The listing builds one solid part. Answer for the finished solid, in the listing's coordinates (mm). A direction names the side the tool comes from. Give positions to 0.01 mm unless a question says otherwise; leave off trailing zeros. Order: outer loops, then holes, each group sorted by start corner. A loop starts at its lowest first (then second) coordinate and runs counter-clockwise, first axis right, second up. Notation, with made-up numbers: (52, 15) - (72, 15) arc R24 ccw to (72, 26) - close; hole circle Ø6 at (21.5, -25.5). An arc over 180 degrees is marked (long way). Answer as a JSON object with one key per item and string values. Group by question number.
Q1. Consider line 1 (Z direction, x = -48, y = 83.75); line 2 (X direction, y = 33, z = 15); line 3 (X direction, y = 79, z = 77). Determine where each line is inside the solid, lowest interval first.
Q2. For faces 4 (the face through (-19, 89, 87)), 5 (the face through (33.289, 86.084, 20.804)), 6 (the face through (-72, 10, 78)), 7 (the face through (-80, 53, 47)), 8 (the face through (-64, 51, 47)), determine the directions among +Z, -Z, +X, -X, +Y, -Y from which every point of the face is accessible in a straight line to the end or side of a thin tool.
Q3. A cutting plane is placed at C-C, the plane y = 11.5. Give the vertices of the cut face in (x, z), and give its area (3 significant figures).
Q4. A cutting plane is placed at B-B, the plane x = 0. Give the vertices of the cut face in (y, z), and give its area (3 significant figures).
Q5. A cutting plane is placed at D-D, the plane x = 48. Give the vertices of the cut face in (y, z), and give its area (3 significant figures).
Q6. A cutting plane is placed at A-A, the plane z = 48. Give the vertices of the cut face in (x, y), and give its area (3 significant figures).
Q7. Given pin 1 (15 mm diameter, centred on x = -1.5, z = 91, fed in from +Y); pin 2 (9.5 mm diameter, centred on y = 86.5, z = 43.5, fed in from +X); pin 3 (16 mm diameter, centred on y = 26.5, z = 65.5, fed in from +X); pin 4 (6 mm diameter, centred on y = 89, z = 56.5, fed in from -X), each flat-ended and moving along its own axis, determine where each tip first touches the part or whether it passes through.
Q8. The mould has two halves that part along X. Classify faces 1 (the face through (-12, 77, 96)), 2 (the face through (-65.703, 78.014, 47.328)), 3 (the face through (-19, 89, 10)): released by +X, released by -X, zero draft, split by the parting line, or undercut.
from build123d import *

# Parameters (mm, degrees)
BRIDGE_BODY_DEPTH          = 96
ARCH_RELIEF_CUT_DEPTH      = 209.038457983
TOP_CHANNEL_SKETCH_W       = 38
TOP_CHANNEL_SKETCH_H       = 96
TOP_CHANNEL_38X6_DEPTH     = 6
CENTER_BORE_SKETCH_R       = 15
CENTER_BORE_30_DEPTH       = 152.69706655
MOUNTING_HOLES_SKETCH_R    = 6
MOUNTING_HOLES_4X_12_DEPTH = 156.17731793
CENTER_POCKET_58X70_DEPTH  = 12


with BuildPart() as part:
    # Bridge Profile Sketch → Bridge Body (new body)
    with BuildSketch(Plane.XY):
        with BuildLine():
            Line((-80, 0), (-64, 0))
            Line((-64, 0), (-64, 54))
            ThreePointArc((-64, 54), (-58.142135624, 68.142135624), (-44, 74))
            Line((-44, 74), (44, 74))
            ThreePointArc((44, 74), (58.142135624, 68.142135624), (64, 54))
            Line((64, 54), (64, 0))
            Line((64, 0), (80, 0))
            Line((80, 0), (80, 72))
            ThreePointArc((80, 72), (65.857864376, 77.857864376), (60, 92))
            Line((60, 92), (-60, 92))
            ThreePointArc((-60, 92), (-65.857864376, 77.857864376), (-80, 72))
            Line((-80, 72), (-80, 0))
        make_face()
    extrude(amount=BRIDGE_BODY_DEPTH)

    # Arch Relief Sketch → Arch Relief Cut (cut, through all)
    with BuildSketch(Plane(origin=(80, 0, 0), x_dir=(0, 0, -1), z_dir=(1, 0, 0))):
        with BuildLine():
            Line((-78, 20), (-78, 0))
            Line((-78, 0), (-18, 0))
            Line((-18, 0), (-18, 20))
            ThreePointArc((-18, 20), (-48, 50), (-78, 20))
        make_face()
    extrude(amount=-ARCH_RELIEF_CUT_DEPTH, mode=Mode.SUBTRACT)

    # Top Channel Sketch → Top Channel 38x6 (cut)
    with BuildSketch(Plane(origin=(0, 92, 0), x_dir=(1, 0, 0), z_dir=(0, 1, 0))):
        with Locations((0, -48)):
            Rectangle(TOP_CHANNEL_SKETCH_W, TOP_CHANNEL_SKETCH_H)
    extrude(amount=-TOP_CHANNEL_38X6_DEPTH, mode=Mode.SUBTRACT)

    # Center Bore Sketch → Center Bore Ø30 (cut, through all)
    with BuildSketch(Plane(origin=(0, 86, 0), x_dir=(1, 0, 0), z_dir=(0, 1, 0))):
        with Locations(Location((0, -48, 0), (0, 0, 270))):
            Circle(CENTER_BORE_SKETCH_R)
    extrude(amount=-CENTER_BORE_30_DEPTH, mode=Mode.SUBTRACT)

    # Mounting Holes Sketch → Mounting Holes 4xØ12 (cut, through all)
    with BuildSketch(Plane(origin=(0, 92, 0), x_dir=(1, 0, 0), z_dir=(0, 1, 0))):
        with Locations(Location((-48, -19, 0), (0, 0, 270))):
            Circle(MOUNTING_HOLES_SKETCH_R)
        with Locations(Location((48, -19, 0), (0, 0, 270))):
            Circle(MOUNTING_HOLES_SKETCH_R)
        with Locations(Location((48, -77, 0), (0, 0, 270))):
            Circle(MOUNTING_HOLES_SKETCH_R)
        with Locations(Location((-48, -77, 0), (0, 0, 270))):
            Circle(MOUNTING_HOLES_SKETCH_R)
    extrude(amount=-MOUNTING_HOLES_4X_12_DEPTH, mode=Mode.SUBTRACT)

    # Center Pocket Sketch → Center Pocket 58x70 (cut)
    with BuildSketch(Plane(origin=(0, 92, 0), x_dir=(1, 0, 0), z_dir=(0, 1, 0))):
        with BuildLine():
            Line((-29, -77), (29, -77))
            ThreePointArc((29, -77), (33.242640687, -75.242640687), (35, -71))
            Line((35, -71), (35, -25))
            ThreePointArc((35, -25), (33.242640687, -20.757359313), (29, -19))
            Line((29, -19), (-29, -19))
            ThreePointArc((-29, -19), (-33.242640687, -20.757359313), (-35, -25))
            Line((-35, -25), (-35, -71))
            ThreePointArc((-35, -71), (-33.242640687, -75.242640687), (-29, -77))
        make_face()
    extrude(amount=-CENTER_POCKET_58X70_DEPTH, mode=Mode.SUBTRACT)


solid = part.part
Reply:
{
 "1": {"line 1": "z = 0 to 13, 25 to 71, 83 to 96", "line 2": "x = -80 to -64, 64 to 80", "line 3": "x = -64.8 to -54, -42 to 42, 54 to 64.8"},
 "2": {"face 4": "+Z, -Z, +Y", "face 5": "+Y", "face 6": "+X, -X, -Y", "face 7": "+Z, -Z, -X, +Y, -Y", "face 8": "+Z, -Z, -Y"},
 "3": {"outline": "(-80, 0) - (-64, 0) - (-64, 18) - (-80, 18) - close; (-80, 78) - (-64, 78) - (-64, 96) - (-80, 96) - close; (64, 0) - (80, 0) - (80, 18) - (64, 18) - close; (64, 78) - (80, 78) - (80, 96) - (64, 96) - close", "area": "1,150 mm^2"},
 "4": {"outline": "(74, 0) - (86, 0) - (86, 19) - (80, 19) - (80, 33) - (74, 33) - close; (74, 63) - (80, 63) - (80, 77) - (86, 77) - (86, 96) - (74, 96) - close", "area": "624 mm^2"},
 "5": {"outline": "(73.6, 0) - (92, 0) - (92, 13) - (73.6, 13) - close; (73.6, 25) - (92, 25) - (92, 71) - (73.6, 71) - close; (73.6, 83) - (92, 83) - (92, 96) - (73.6, 96) - close", "area": "1,330 mm^2"},
 "6": {"outline": "(-80, 50) - (-64, 50) - (-64, 54) arc R20 cw to (-44, 74) - (-15, 74) - (-15, 80) - (-35, 80) - (-35, 92) - (-60, 92) arc R20 cw to (-80, 72) - close; (15, 74) - (44, 74) arc R20 cw to (64, 54) - (64, 50) - (80, 50) - (80, 72) arc R20 cw to (60, 92) - (35, 92) - (35, 80) - (15, 80) - close", "area": "2,170 mm^2"},
 "7": {"pin 1": "stops at y = 86", "pin 2": "stops at x = 62.83", "pin 3": "passes through", "pin 4": "stops at x = -60.92"},
 "8": {"face 1": "zero draft", "face 2": "released by -X", "face 3": "undercut"}
}
